Geometry check sheet. Reference: the model listing, model coordinates, mm. A direction names the side the tool comes from. Round coordinates to 2 decimals unless told otherwise and drop trailing zeros. Order: outer loops, then holes, each group sorted by start corner. A loop starts at its lowest first (then second) coordinate and runs counter-clockwise, first axis right, second up.
(1) Sectioned sample at C-C (z = 17.5). Record the boundary of the cut face in (x, y), plus the area to 3 significant figures.
(2) Sectioned sample at B-B (x = 0). Record the boundary of the cut face in (y, z), plus the area to 3 significant figures.
(3) Sectioned sample at D-D (y = 259). Record the boundary of the cut face in (x, z), plus the area to 3 significant figures.
(4) Release check for a two-part mould opening along Y. For faces 1 (the face through (0, 312, 0)), 2 (the face through (-22.94, 129.96, -24.54)), 3 (the face through (-7.97, 3.04, -4.71)) record: +Y half, -Y half, draft (parallel to the pull), parting line (faces both ways), or undercut.
(5) Go/stop test with flat-tipped pins: pin 1 (23 mm diameter, centred on x = 0, y = 156, fed in from +Z); pin 2 (5.5 mm diameter, centred on x = 10, z = 17.5, fed in from +Y); pin 3 (3 mm diameter, centred on x = 26.5, z = -24.5, fed in from +Y); pin 4 (3 mm diameter, centred on x = 24.5, z = -26, fed in from -Y). Record where each tip stops, or that it passes through.
(6) Material ranges on line 1 along X through (y, z) = (2.35, 17.5); line 2 along X through (y, z) = (132.5, -22.9); line 3 along Y through (x, z) = (12, -15), recorded low to high.
(7) Set-up check for faces 4 (the face through (27, 191, -25)), 5 (the face through (16, 158, -21.5)), 6 (the face through (27, 121, -25)): record each of +Z, -Z, +X, -X, +Y, -Y from which the full face is reachable in a straight line by a thin tool's end or side.
(8) Sectioned sample at A-A (z = -15). Record the boundary of the cut face in (x, y).
from build123d import *

# Parameters (mm, degrees)
SKETCH_1_W          = 38
SKETCH_1_H          = 55
EXTRUDE_1_DEPTH     = 6
SKETCH_2_R          = 3
CUT_EXTRUDE_1_DEPTH = 16
SKETCH_3_W          = 38
SKETCH_3_H          = 6
EXTRUDE_2_DEPTH     = 300
EXTRUDE_START       = 6
SKETCH_5_R          = 3
EXTRUDE_3_DEPTH     = 6
SKETCH_6_W          = 70
SKETCH_6_H          = 70
EXTRUDE_4_DEPTH     = 6
SKETCH_7_R          = 2.6
SKETCH_7_R_2        = 10
CUT_EXTRUDE_2_DEPTH = 10


with BuildPart() as part:
    # 草图1 → 凸台-拉伸1 (new body)
    with BuildSketch(Plane(origin=(0, 0, 0), x_dir=(1, 0, 0), z_dir=(0, 1, 0))):
        Rectangle(SKETCH_1_W, SKETCH_1_H)
    extrude(amount=EXTRUDE_1_DEPTH)

    # 草图2 → 切除-拉伸1 (cut)
    with BuildSketch(Plane(origin=(0, 6, 0), x_dir=(1, 0, 0), z_dir=(0, 1, 0))):
        with Locations(Location((-10, 2.5, 0), (0, 0, 270))):
            Circle(SKETCH_2_R)
        with Locations(Location((10, 2.5, 0), (0, 0, 270))):
            Circle(SKETCH_2_R)
        with Locations(Location((10, -17.5, 0), (0, 0, 270))):
            Circle(SKETCH_2_R)
        with Locations(Location((-10, -17.5, 0), (0, 0, 270))):
            Circle(SKETCH_2_R)
    extrude(amount=-CUT_EXTRUDE_1_DEPTH, mode=Mode.SUBTRACT)

    # 草图3 → 凸台-拉伸2 (add)
    with BuildSketch(Plane(origin=(0, 6, 0), x_dir=(1, 0, 0), z_dir=(0, 1, 0))):
        with Locations((0, 24.5)):
            Rectangle(SKETCH_3_W, SKETCH_3_H)
    extrude(amount=EXTRUDE_2_DEPTH)

    # 草图5 → 凸台-拉伸3 (add)
    with BuildSketch(Plane(origin=(0, 306, 0), x_dir=(1, 0, 0), z_dir=(0, 1, 0)).offset(EXTRUDE_START)):
        Polygon((-19, 27.5), (-19, 21.5), (-19, -27.5), (19, -27.5), (19, 21.5), (19, 27.5), align=None)
        with Locations(Location((-10, 2.5, 0), (0, 0, 270))):
            Circle(SKETCH_5_R, mode=Mode.SUBTRACT)
        with Locations(Location((10, 2.5, 0), (0, 0, 270))):
            Circle(SKETCH_5_R, mode=Mode.SUBTRACT)
        with Locations(Location((-10, -17.5, 0), (0, 0, 270))):
            Circle(SKETCH_5_R, mode=Mode.SUBTRACT)
        with Locations(Location((10, -17.5, 0), (0, 0, 270))):
            Circle(SKETCH_5_R, mode=Mode.SUBTRACT)
    extrude(amount=-EXTRUDE_3_DEPTH)

    # 草图6 → 凸台-拉伸4 (add)
    with BuildSketch(Plane(origin=(0, 0, -27.5), x_dir=(-1, 0, 0), z_dir=(0, 0, -1))):
        with Locations((0, 156)):
            Rectangle(SKETCH_6_W, SKETCH_6_H)
    extrude(amount=-EXTRUDE_4_DEPTH)

    # 草图7 → 切除-拉伸2 (cut)
    with BuildSketch(Plane(origin=(0, 0, -27.5), x_dir=(-1, 0, 0), z_dir=(0, 0, -1))):
        with Locations((23.545, 179.545)):
            Circle(SKETCH_7_R)
        with Locations((23.5, 132.5)):
            Circle(SKETCH_7_R)
        with Locations((-23.5, 132.5)):
            Circle(SKETCH_7_R)
        with Locations((-23.545, 179.545)):
            Circle(SKETCH_7_R)
        with Locations((0, 156)):
            Circle(SKETCH_7_R_2)
    extrude(amount=-CUT_EXTRUDE_2_DEPTH, mode=Mode.SUBTRACT)


solid = part.part
Answer below:
1. outline: (-19, 0) - (-13, 0) - (-13, 6) - (-19, 6) - close; (-19, 306) - (-13, 306) - (-13, 312) - (-19, 312) - close; (-7, 0) - (7, 0) - (7, 6) - (-7, 6) - close; (-7, 306) - (7, 306) - (7, 312) - (-7, 312) - close; (13, 0) - (19, 0) - (19, 6) - (13, 6) - close; (13, 306) - (19, 306) - (19, 312) - (13, 312) - close
1. area: 312 mm2
2. outline: (0, -27.5) - (146, -27.5) - (146, -21.5) - (6, -21.5) - (6, 27.5) - (0, 27.5) - close; (166, -27.5) - (312, -27.5) - (312, 27.5) - (306, 27.5) - (306, -21.5) - (166, -21.5) - close
2. area: 2,340 mm2
3. outline: (-19, -27.5) - (19, -27.5) - (19, -21.5) - (-19, -21.5) - close
3. area: 228 mm2
4. face 1: +Y half
4. face 2: undercut
4. face 3: draft
5. pin 1: stops at z = -21.5
5. pin 2: passes through
5. pin 3: stops at y = 191
5. pin 4: stops at y = 121
6. line 1: x = -19 to -13, -7 to 7, 13 to 19
6. line 2: x = -35 to -26.1, -20.9 to 20.9, 26.1 to 35
6. line 3: y = 0 to 6, 306 to 312
7. face 4: +Z, -Z, +X, +Y
7. face 5: +Z, +X, -X
7. face 6: +Z, -Z, +X, -Y
8. outline: (-19, 0) - (19, 0) - (19, 6) - (-19, 6) - close; (-19, 306) - (19, 306) - (19, 312) - (-19, 312) - close
